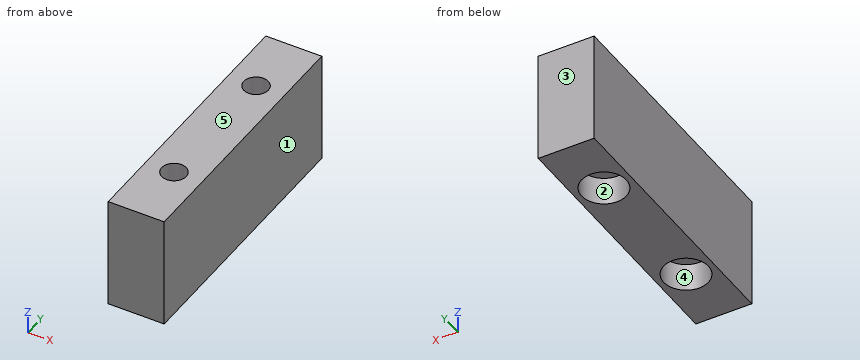
```python
from build123d import *

# Parameters (mm, degrees)
SKETCH_1_W                = 20
SKETCH_1_H                = 48
EXTRUDE_1_DEPTH           = 10
HOLE_WIZARD_1_D           = 4.4
HOLE_WIZARD_1_CBORE_D     = 8
HOLE_WIZARD_1_CBORE_DEPTH = 5


with BuildPart() as part:
    # 草图1 → 凸台-拉伸1 (new body)
    with BuildSketch(Plane(origin=(0, 0, 0), x_dir=(0, 0, -1), z_dir=(1, 0, 0))):
        Rectangle(SKETCH_1_W, SKETCH_1_H)
    extrude(amount=EXTRUDE_1_DEPTH)

    # 打孔尺寸(%根据)内六角圆柱头螺钉的类型1 (through all)
    with Locations(Plane(origin=(0, 0, -10), x_dir=(-1, 0, 0), z_dir=(0, 0, -1))):
        with Locations((-5, -12.5), (-5, 12.5)):
            CounterBoreHole(HOLE_WIZARD_1_D / 2, HOLE_WIZARD_1_CBORE_D / 2, HOLE_WIZARD_1_CBORE_DEPTH)


solid = part.part
```
For this review, take the finished solid that the model builds, in its own axes (mm). Face numbers are marked on the shaded views. A direction names the side the tool comes from. Give positions to 0.01 mm unless a question says otherwise; leave off trailing zeros. Order: outer loops, then holes, each group sorted by start corner. A loop starts at its lowest first (then second) coordinate and runs counter-clockwise, first axis right, second up.
1) For the marked faces 4 and 5, list the 3-axis set-ups (+Z, -Z, +X, -X, +Y, -Y) from which the entire face can be reached by the end or side of a thin tool; tool diameter is ignored.
2) The part is to be moulded in two halves that separate along X. For the marked faces 1, 2 and 3, say which applies: released by +X, released by -X, zero draft, split by the parting line, or undercut.
3) Take a section at D-D (x = 1.5). Give the boundary of the cut face in (y, z).
4) Wall thickness on line 1 (Y direction, x = 5, z = -6.2); line 2 (Y direction, x = 5, z = 4); line 3 (Z direction, x = 2.25, y = 13): over which ranges is each line inside the solid? List them lowest first.
5) Take a section at C-C (x = 5). Give the boundary of the cut face in (y, z).
6) Take a section at B-B (y = -12.5). Give the boundary of the cut face in (x, z), then the cut area to 3 significant figures.
7) Take a section at A-A (z = -3.5). Give the boundary of the cut face in (x, y), then the cut area to 3 significant figures.
Derived:
1. face 4: -Z
1. face 5: +Z, +X, -X, +Y, -Y
2. face 1: released by +X
2. face 2: undercut
2. face 3: zero draft
3. outline: (-24, -10) - (-14.44, -10) - (-14.44, -5) - (-10.56, -5) - (-10.56, -10) - (10.56, -10) - (10.56, -5) - (14.44, -5) - (14.44, -10) - (24, -10) - (24, 10) - (-24, 10) - close
4. line 1: y = -24 to -16.5, -8.5 to 8.5, 16.5 to 24
4. line 2: y = -24 to -14.7, -10.3 to 10.3, 14.7 to 24
4. line 3: z = -5 to 10
5. outline: (-24, -10) - (-16.5, -10) - (-16.5, -5) - (-14.7, -5) - (-14.7, 10) - (-24, 10) - close; (-10.3, -5) - (-8.5, -5) - (-8.5, -10) - (8.5, -10) - (8.5, -5) - (10.3, -5) - (10.3, 10) - (-10.3, 10) - close; (14.7, -5) - (16.5, -5) - (16.5, -10) - (24, -10) - (24, 10) - (14.7, 10) - close
6. outline: (0, -10) - (1, -10) - (1, -5) - (2.8, -5) - (2.8, 10) - (0, 10) - close; (7.2, -5) - (9, -5) - (9, -10) - (10, -10) - (10, 10) - (7.2, 10) - close
6. area: 94.0 mm2
7. outline: (0, -24) - (10, -24) - (10, 24) - (0, 24) - close; hole circle Ø4.4 at (5, -12.5); hole circle Ø4.4 at (5, 12.5)
7. area: 450 mm2
